Input: part model. Units: mm. Frame: model coordinates. A direction names the side the tool comes from. Give positions to 0.01 mm unless a question says otherwise; leave off trailing zeros. Loops run counter-clockwise (first coordinate to the right, second up) from the corner with the lowest first, then second, coordinate; pieces in that order, holes last. Notation, with made-up numbers: (76, -11.5) -> (127, -11.5) arc R26 cw to (127, 16.5) -> close; hole circle Ø8 at (-2, 13). An arc over 180 degrees is marked (long way). Answer as a JSON object with one key per item and string values.
```python
from build123d import *

# Parameters (mm, degrees)
BOSS_EXTRUDE1_DEPTH       = 20
CHAMFER1_SIZE             = 2
M8X1_0_TAPPED_HOLE1_D     = 7
M8X1_0_TAPPED_HOLE1_DEPTH = 13
M8X1_0_TAPPED_HOLE1_TIP   = 2.103012167
HOLE2_D                   = 9
SKETCH15_R                = 32.5
CUT_EXTRUDE3_DEPTH        = 2.5
CUT_EXTRUDE4_START        = -2.5
SKETCH16_R                = 32.5
CUT_EXTRUDE4_DEPTH        = 2.5
HOLE3_D                   = 4


with BuildPart() as part:
    # Sketch1 → Boss-Extrude1 (new body)
    with BuildSketch(Plane.XY):
        with BuildLine():
            Line((-50, 24), (-33, 24))
            Line((-33, 24), (-33, 47))
            Line((-33, 47), (33, 47))
            Line((33, 47), (33, 24))
            Line((33, 24), (50, 24))
            Line((50, 24), (50, 0))
            Line((50, 0), (30, 0))
            ThreePointArc((30, 0), (0, 30), (-30, 0))
            Line((-30, 0), (-50, 0))
            Line((-50, 0), (-50, 24))
        make_face()
    extrude(amount=BOSS_EXTRUDE1_DEPTH)

    # Chamfer1
    chamfer1_edges = [part.edges().sort_by_distance(p)[0] for p in [
        (-50, 24, 10),
        (-33, 47, 10),
        (33, 47, 10),
        (50, 24, 10),
    ]]
    chamfer(chamfer1_edges, length=CHAMFER1_SIZE)

    # M8x1.0 Tapped Hole1
    with Locations(Plane(origin=(0, 47, 0), x_dir=(1, 0, 0), z_dir=(0, 1, 0))):
        with Locations((0, -10)):
            Hole(M8X1_0_TAPPED_HOLE1_D / 2, depth=M8X1_0_TAPPED_HOLE1_DEPTH)
            with Locations((0, 0, -(M8X1_0_TAPPED_HOLE1_DEPTH + M8X1_0_TAPPED_HOLE1_TIP / 2))):  # 118° drill point
                Cone(0, M8X1_0_TAPPED_HOLE1_D / 2, M8X1_0_TAPPED_HOLE1_TIP, mode=Mode.SUBTRACT)

    # Hole2 (through all)
    with Locations(Plane(origin=(0, 24, 0), x_dir=(1, 0, 0), z_dir=(0, 1, 0))):
        with Locations((-41, -10), (41, -10)):
            Hole(HOLE2_D / 2)

    # Sketch15 → Cut-Extrude3 (cut)
    with BuildSketch(Plane(origin=(0, 0, 0), x_dir=(-1, 0, 0), z_dir=(0, 0, -1))):
        Circle(SKETCH15_R)
    extrude(amount=-CUT_EXTRUDE3_DEPTH, mode=Mode.SUBTRACT)

    # Sketch16 → Cut-Extrude4 (cut)
    with BuildSketch(Plane.XY.offset(20).offset(CUT_EXTRUDE4_START)):
        Circle(SKETCH16_R)
    extrude(amount=CUT_EXTRUDE4_DEPTH, mode=Mode.SUBTRACT)

    # Hole3 (through all)
    with Locations(Plane(origin=(0, 47, 0), x_dir=(1, 0, 0), z_dir=(0, 1, 0))):
        with Locations((0, -10)):
            Hole(HOLE3_D / 2)


solid = part.part
```
Q1. Pin query (flat end, axial travel): pin 1 (6.5 mm diameter, centred on x = 0, z = 10, fed in from -Y); pin 2 (5 mm diameter, centred on y = 33, z = 11.5, fed in from +X); pin 3 (10 mm diameter, centred on x = -12.5, z = 5.5, fed in from -Y). Return the tip coordinate at first contact, or that it passes through.
Evaluation:
{"pin 1": "stops at y = 29.82", "pin 2": "stops at x = 33", "pin 3": "stops at y = 24.37"}
Q2. Section A-A, the plane y = 16.5. Return the cut outline in (x, z), then the cut area to 3 significant figures.
Evaluation:
{"outline": "(-50, 0) -> (-28, 0) -> (-28, 2.5) -> (-25.05, 2.5) -> (-25.05, 17.5) -> (-28, 17.5) -> (-28, 20) -> (-50, 20) -> close; (25.05, 2.5) -> (28, 2.5) -> (28, 0) -> (50, 0) -> (50, 20) -> (28, 20) -> (28, 17.5) -> (25.05, 17.5) -> close; hole circle Ø9 at (-41, 10); hole circle Ø9 at (41, 10)", "area": "841 mm2"}
Q3. Section B-B, the plane x = 0. Return the cut outline in (y, z).
Evaluation:
{"outline": "(30, 2.5) -> (32.5, 2.5) -> (32.5, 0) -> (47, 0) -> (47, 6.5) -> (34, 6.5) -> (33.1, 8) -> (30, 8) -> close; (30, 12) -> (33.1, 12) -> (34, 13.5) -> (47, 13.5) -> (47, 20) -> (32.5, 20) -> (32.5, 17.5) -> (30, 17.5) -> close"}
Q4. Section C-C, the plane z = 10. Give the number of separate pieces and of enclosed holes in the cut face, then the cut area to 3 significant figures.
Evaluation:
{"separate pieces": "4", "enclosed holes": "0", "area": "1,960 mm2"}
Q5. Draft query along X for faces 1 (the flat face through (1, 34, 20)), 2 (the cylindrical face through (-45.292, 11.832, 8.648)), 3 (the flat face through (49, 23, 10)), 4 (the cylindrical face through (0.66, 29.993, 6.562)). Return one class per face: +X half, -X half, draft (parallel to the pull), parting line (faces both ways), or undercut.
Evaluation:
{"face 1": "draft", "face 2": "undercut", "face 3": "+X half", "face 4": "undercut"}
Q6. Access query for faces 5 (the flat face through (0, 31, 17.5)), 6 (the cylindrical face through (0.759, 40.409, 13.417)), 7 (the flat face through (40, 24, 5)), 8 (the flat face through (-33, 34, 10)), 9 (the flat face through (0, 31, 2.5)). Directions: +Z, -Z, +X, -X, +Y, -Y. A direction counts if a zero-diameter tool reaches every point of the face in a straight line with its end or side. Return the directions, or none.
Evaluation:
{"face 5": "+Z, -Y", "face 6": "+Y", "face 7": "+Z, -Z, +X, +Y", "face 8": "+Z, -Z, -X, +Y", "face 9": "-Z, -Y"}
Q7. Section D-D, the plane y = 39. Return the cut outline in (x, z), then the cut area to 3 significant figures.
Evaluation:
{"outline": "(-33, 0) -> (33, 0) -> (33, 20) -> (-33, 20) -> close; hole circle Ø7 at (0, 10)", "area": "1,280 mm2"}
Q8. Ray query, line 1 along X through (y, z) = (37, 10); line 2 along Z through (x, y) = (41, 10.25); line 3 along X through (y, z) = (33.5, 11.75). Return the intervals inside material, ascending.
Evaluation:
{"line 1": "x = -33 to -3.5, 3.5 to 33", "line 2": "z = 0 to 5.5, 14.5 to 20", "line 3": "x = -33 to -2.01, 2.01 to 33"}
